```python
from build123d import *

# Parameters (mm, degrees)
BOSS_EXTRUDE1_DEPTH            = 5
F_2_5_2_5_DIAMETER_HOLE1_D     = 2.5
F_2_5_2_5_DIAMETER_HOLE1_DEPTH = 31.642263263
CHAMFER1_SIZE                  = 0.5


with BuildPart() as part:
    # Sketch1 → Boss-Extrude1 (new body)
    with BuildSketch(Plane(origin=(14.029336503, -7.536520805, 0), x_dir=(0.4732361692035663, 0.8809355981895235, 0), z_dir=(0.8809355981895235, -0.4732361692035663, -1.915856770880308e-15))):
        with BuildLine():
            Line((-90.390644299, -267.73860401), (-32.919543007, -250.502812288))
            ThreePointArc((-32.919543007, -250.502812288), (-31.243071775, -247.390025079), (-34.355858984, -245.713553847))
            Line((-34.355858984, -245.713553847), (-91.826960276, -262.949345569))
            ThreePointArc((-91.826960276, -262.949345569), (-93.503431508, -266.062132778), (-90.390644299, -267.73860401))
        make_face()
    extrude(amount=-BOSS_EXTRUDE1_DEPTH)

    # Sketch2 → Revolve1 (revolve)
    with BuildSketch(Plane.XY.offset(-265.34397479)):
        Polygon((-37.304454842, -81.963976858), (-37.896000054, -83.065146356), (-33.491322063, -85.431327202), (-32.899776851, -84.330157704), align=None)
    revolve(axis=Axis((-36.90956153, -83.595058405, -265.34397479), (0.880935598189524, -0.47323616920356526, 0)))

    # Sketch3 → Revolve2 (revolve)
    with BuildSketch(Plane.XY.offset(-265.34397479)):
        Polygon((-28.49509886, -86.69633855), (-29.086644072, -87.797508048), (-24.681966081, -90.163688894), (-24.090420869, -89.062519396), align=None)
    revolve(axis=Axis((-28.100205548, -88.327420097, -265.34397479), (0.8809355981895229, -0.4732361692035673, 0)))

    # Ø2.5 (2.5) Diameter Hole1
    with Locations(Plane(origin=(9.624658513, -5.170339959, 0), x_dir=(0, 0, 1), z_dir=(-0.8809355981895236, 0.4732361692035664, 1.9158567708803085e-15))):
        with Locations((-248.108183067, -33.637700995)):
            Hole(F_2_5_2_5_DIAMETER_HOLE1_D / 2, depth=F_2_5_2_5_DIAMETER_HOLE1_DEPTH)

    # Chamfer1
    chamfer1_edges = [part.edges().sort_by_distance(p)[0] for p in [
        (-5.160693088, -32.693474082, -247.390025079),
        (-20.23247849, -60.749808642, -254.331449708),
        (-34.624547222, -87.540841327, -266.062132778),
        (-15.827800499, -63.115989488, -254.331449708),
        (-0.756015097, -35.059654928, -247.390025079),
        (-15.148083829, -61.850687613, -259.120708149),
        (-30.219869231, -89.907022173, -266.062132778),
        (-19.55276182, -59.484506767, -259.120708149),
    ]]
    chamfer(chamfer1_edges, length=CHAMFER1_SIZE)


solid = part.part
```
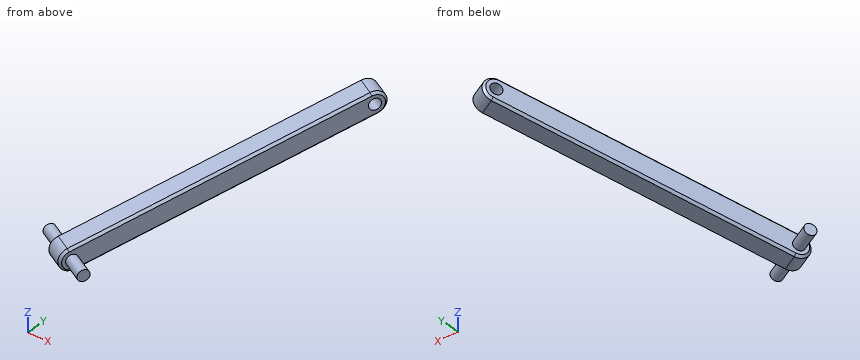
Verification items for the finished model (mm, model axes). Coordinates: 2 decimals unless noted, no trailing zeros. Write each loop counter-clockwise with the first axis right and the second up, starting at its lowest first coordinate (ties: lowest second). Pieces come first, ordered by that corner, then holes. Notation, with made-up numbers: M -22,35.5 L -14,35.5 A14 cw -14,48.5 Z; hole C -17.5,13.5 d11. An arc over 180 degrees is marked long. Answer as a JSON object with one key per item and string values. Group by question number.
(1) Cross-section at A-A, the plane x = -18.5. Record the cut outline in (y, z).
(2) Material ranges on line 1 (Y direction, x = -3.5, z = -250); line 2 (Z direction, x = -22, y = -68); line 3 (Z direction, x = -27, y = -75), recorded low to high.
(3) Gauge pin test, flat ends, axial feed: pin 1 (3 mm diameter, centred on x = -8, z = -249, fed in from -Y); pin 2 (10 mm diameter, centred on x = -31, z = -250, fed in from +Y); pin 3 (3 mm diameter, centred on x = -26, z = -261, fed in from -Y). Record the tip position at first contact, or that the pin passes through.
(4) Cross-section at B-B, the plane y = -54. Record the cut outline in (x, z), and give its area (3 significant figures).
Reply:
{
 "1": {"outline": "M -68.09,-260.72 L -67.03,-260.97 L -58.58,-258.73 L -57.52,-257.93 L -57.52,-253.76 L -58.58,-253.51 L -67.03,-255.75 L -68.09,-256.55 Z"},
 "2": {"line 1": "-40.17 to -34.45", "line 2": "-261.72 to -256.5", "line 3": "-264.28 to -259.06"},
 "3": {"pin 1": "y = -49.87", "pin 2": "through", "pin 3": "y = -84.12"},
 "4": {"outline": "M -16.61,-256.73 L -16.04,-257.17 L -11.5,-256.53 L -10.93,-255.93 L -10.93,-251.75 L -11.5,-251.31 L -16.04,-251.95 L -16.61,-252.56 Z", "area": "29.0 mm²"}
}
